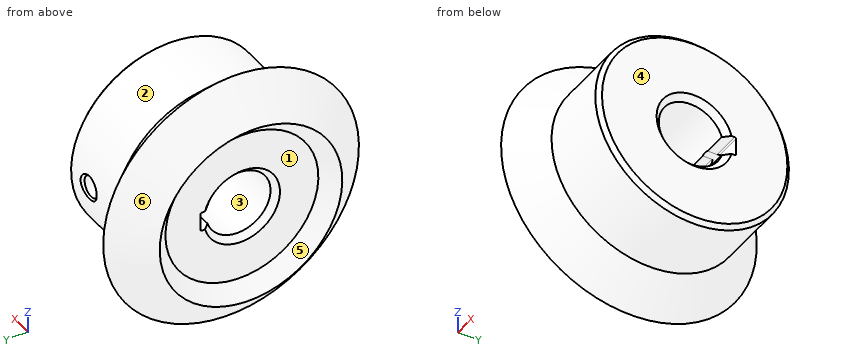
from build123d import *

# Parameters (mm, degrees)
CUT_EXTRUDE_1_DEPTH = 21.26


with BuildPart() as part:
    # 草图1 → 旋转1 (revolve)
    with BuildSketch(Plane.XY, mode=Mode.PRIVATE) as revolve_1_sk:
        Polygon((-21.26, 14.14569447), (-19, 11.85), (-19, 5), (0, 5), (0, 14.363603897), (-0.636396103, 15), (-11.5, 15), (-16.31, 19.81), align=None)
    revolve(revolve_1_sk.sketch.rotate(Axis((0, 0, 0), (-1, 0, 0)), 270), axis=Axis((0, 0, 0), (-1, 0, 0)))

    # 草图2 → 切除-旋转1 (revolve, cut)
    with BuildSketch(Plane.XY, mode=Mode.PRIVATE) as cut_revolve_1_sk:
        Polygon((-19, 0), (-19, 5.9), (-18.1, 5), (-0.9, 5), (0, 5.9), (0, 0), align=None)
    revolve(cut_revolve_1_sk.sketch.rotate(Axis((0, 0, 0), (-1, 0, 0)), 270), axis=Axis((0, 0, 0), (-1, 0, 0)), mode=Mode.SUBTRACT)

    # 草图3 → 切除-旋转2 (revolve, cut)
    with BuildSketch(Plane(origin=(-5, 0, 0), x_dir=(0, 0, -1), z_dir=(1, 0, 0)), mode=Mode.PRIVATE) as cut_revolve_2_sk:
        Polygon((0, 15), (2, 15), (1.621, 14.621), (1.621, 4.582575695), (0, 4.582575695), align=None)
    revolve(cut_revolve_2_sk.sketch.rotate(Axis((-5, 4.582575695, 0), (0, 1, 0)), 180), axis=Axis((-5, 4.582575695, 0), (0, 1, 0)), mode=Mode.SUBTRACT)

    # 草图4 → 切除-拉伸1 (cut)
    with BuildSketch(Plane(origin=(0, 0, 0), x_dir=(0, 0, -1), z_dir=(1, 0, 0))):
        with BuildLine():
            Line((-1.5, 0), (1.5, 0))
            Line((1.5, 0), (1.5, 6.2))
            ThreePointArc((1.5, 6.2), (1.441421356, 6.341421356), (1.3, 6.4))
            Line((1.3, 6.4), (-1.3, 6.4))
            ThreePointArc((-1.3, 6.4), (-1.441421356, 6.341421356), (-1.5, 6.2))
            Line((-1.5, 6.2), (-1.5, 0))
        make_face()
    extrude(amount=-CUT_EXTRUDE_1_DEPTH, mode=Mode.SUBTRACT)


solid = part.part
Geometry check sheet. Reference: the model listing, model coordinates, mm. Face numbers are marked on the shaded views. A direction names the side the tool comes from. Round coordinates to 2 decimals unless told otherwise and drop trailing zeros. Write each loop counter-clockwise with the first axis right and the second up, starting at its lowest first coordinate (ties: lowest second). Pieces come first, ordered by that corner, then holes. Notation, with made-up numbers: (79.25, 3.5) -> (110.25, 3.5) arc R22 cw to (110.25, 16.5) -> close; hole circle Ø11 at (86, -15.5). An arc over 180 degrees is marked (long way). One line per item, written item: value. Start each with the question number.
(1) Cross-section at A-A, the plane y = 0. Record the cut outline in (x, z), and give its area (3 significant figures).
(2) Access from +Z, -Z, +X, -X, +Y, -Y to the whole of each face (thin tool, end or side, straight path). Record for the marked faces 1, 2 and 3.
(3) Scan lines: line 1 (Z direction, x = -10.5, y = 1.5); line 2 (X direction, y = 0, z = 10); line 3 (X direction, y = 7.5, z = 0). Record each from-to range of solid material in increasing order. Write a range as [from, to].
(4) Cross-section at C-C, the plane x = -15.5. Record the cut outline in (y, z), and give its area (3 significant figures).
(5) Go/stop test with flat-tipped pins: pin 1 Ø10 at (y, z) = (-2.5, -11.5) entering from -X; pin 2 Ø8 at (y, z) = (13.5, -14.5) entering from -X; pin 3 Ø1.6 at (x, y) = (-13, 5.5) entering from -Z; pin 4 Ø1.5 at (x, z) = (-15, 8.5) entering from +Y. Record where each tip stops, or that it passes through.
(6) Draft check along Y on the marked faces 4, 5 and 6. Enter one of: +Y half, -Y half, draft (parallel to the pull), parting line (faces both ways), or undercut.
(7) Cross-section at B-B, the plane z = 0. Record the cut outline in (x, y), and give its area (3 significant figures).
(8) Cross-section at D-D, the plane x = -12.25. Record the cut outline in (y, z).
Answer:
1. outline: (-21.26, -14.15) -> (-16.31, -19.81) -> (-11.5, -15) -> (-0.64, -15) -> (0, -14.36) -> (0, -5.9) -> (-0.9, -5) -> (-18.1, -5) -> (-19, -5.9) -> (-19, -11.85) -> close; (-21.26, 14.15) -> (-19, 11.85) -> (-19, 5.9) -> (-18.1, 5) -> (-0.9, 5) -> (0, 5.9) -> (0, 14.36) -> (-0.64, 15) -> (-11.5, 15) -> (-16.31, 19.81) -> close
1. area: 430 mm²
2. face 1: -X
2. face 2: +X
2. face 3: +X, -X
3. line 1: [-14.92, -4.77], [4.77, 14.92]
3. line 2: [-19, 0]
3. line 3: [-19, -6.62], [-3.38, 0]
4. outline: circle Ø38 at (0, 0); hole (4.77, -1.5) -> (6.2, -1.5) arc R0.2 ccw to (6.4, -1.3) -> (6.4, 1.3) arc R0.2 ccw to (6.2, 1.5) -> (4.77, 1.5) arc R5 ccw (long way) to start
4. area: 1,050 mm²
5. pin 1: x = -21.26
5. pin 2: x = -19.8
5. pin 3: z = -16.44
5. pin 4: y = 17.35
6. face 4: draft
6. face 5: undercut
6. face 6: parting line
7. outline: (-21.26, -14.15) -> (-16.31, -19.81) -> (-11.5, -15) -> (-0.64, -15) -> (0, -14.36) -> (0, -5.9) -> (-0.9, -5) -> (-18.1, -5) -> (-19, -5.9) -> (-19, -11.85) -> close; (-21.26, 14.15) -> (-19, 11.85) -> (-19, 6.4) -> (-6.62, 6.4) -> (-6.62, 14.62) -> (-7, 15) -> (-11.5, 15) -> (-16.31, 19.81) -> close; (-3.38, 6.4) -> (0, 6.4) -> (0, 14.36) -> (-0.64, 15) -> (-3, 15) -> (-3.38, 14.62) -> close
7. area: 376 mm²
8. outline: circle Ø31.5 at (0, 0); hole (4.77, -1.5) -> (6.2, -1.5) arc R0.2 ccw to (6.4, -1.3) -> (6.4, 1.3) arc R0.2 ccw to (6.2, 1.5) -> (4.77, 1.5) arc R5 ccw (long way) to start
